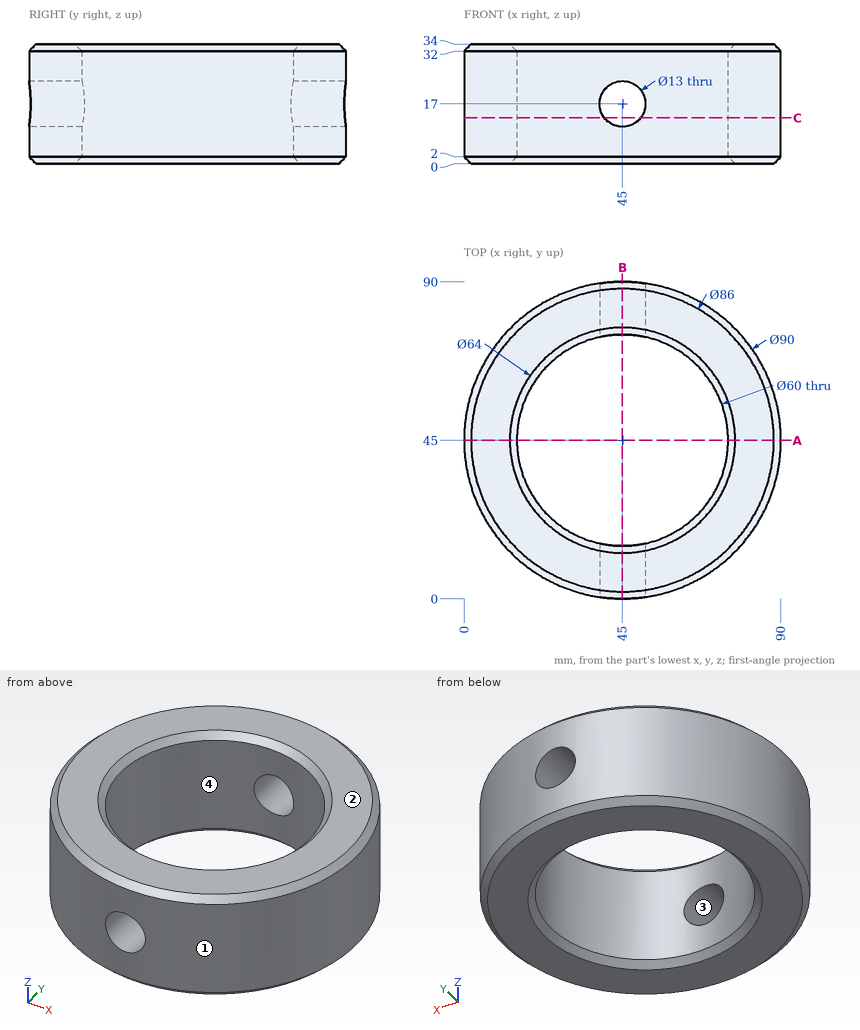
Drawing for the job (mm, zero at the part's lowest x, y, z). Round coordinates to 2 decimals unless told otherwise and drop trailing zeros. Write each loop counter-clockwise with the first axis right and the second up, starting at its lowest first coordinate (ties: lowest second). Pieces come first, ordered by that corner, then holes. Notation, with made-up numbers: (-8, 37) - (4, 37) arc R18 ccw to (4, 58) - close; hole circle Ø5 at (86.25, -30.75). An arc over 180 degrees is marked (long way). Return JSON: item names as keys, results as strings. Group by question number.
Item 1: Mould opens along X. For the marked faces 1, 2, 3 and 4 say: +X half, -X half, draft (parallel to the pull), parting line (faces both ways), or undercut.
Item 2: Flat gauge pins, fed straight in: pin 1 Ø4 at (y, z) = (47.5, 5.5) entering from -X; pin 2 Ø12 at (x, z) = (21, 28) entering from +Y; pin 3 Ø6 at (x, z) = (54, 25) entering from -Y. Where does each tip first touch, or does it go through?
Item 3: Band-saw the part on B-B on x = 45. List the corners of the cut face in (y, z), plus the area to 3 significant figures.
Item 4: Band-saw the part on C-C on z = 13. List the corners of the cut face in (x, y), plus the area to 3 significant figures.
Item 5: Band-saw the part on A-A on y = 45. List the corners of the cut face in (x, z).
Item 6: Probe probe 1 along Y at (x, z) = (45.5, 3); probe 2 along Y at (x, z) = (29.5, 21); probe 3 along X at (y, z) = (59, 22). List the from-to ranges inside material, lowest first.
Resolved:
{
 "1": {"face 1": "parting line", "face 2": "draft", "face 3": "undercut", "face 4": "undercut"},
 "2": {"pin 1": "stops at x = 0", "pin 2": "stops at y = 86.24", "pin 3": "stops at y = 0.4"},
 "3": {"outline": "(0, 2) - (2, 0) - (13, 0) - (15, 2) - (15, 10.5) - (0, 10.5) - close; (0, 23.5) - (15, 23.5) - (15, 32) - (13, 34) - (2, 34) - (0, 32) - close; (75, 2) - (77, 0) - (88, 0) - (90, 2) - (90, 10.5) - (75, 10.5) - close; (75, 23.5) - (90, 23.5) - (90, 32) - (88, 34) - (77, 34) - (75, 32) - close", "area": "614 mm²"},
 "4": {"outline": "(39.88, 0.29) - (39.88, 15.44) arc R30 cw to (39.88, 74.56) - (39.88, 89.71) arc R45 ccw to start; (50.12, 0.29) arc R45 ccw to (50.12, 89.71) - (50.12, 74.56) arc R30 cw to (50.12, 15.44) - close", "area": "3,230 mm²"},
 "5": {"outline": "(0, 2) - (2, 0) - (13, 0) - (15, 2) - (15, 32) - (13, 34) - (2, 34) - (0, 32) - close; (75, 2) - (77, 0) - (88, 0) - (90, 2) - (90, 32) - (88, 34) - (77, 34) - (75, 32) - close"},
 "6": {"probe 1": "y = 0 to 15, 75 to 90", "probe 2": "y = 2.75 to 19.31, 70.69 to 87.25", "probe 3": "x = 2.23 to 18.47, 71.53 to 87.77"}
}
